Job drawing, mm, ordinate dimensions from the low corner. One solid piece. A direction names the side the tool comes from. Give positions to 0.01 mm unless a question says otherwise; leave off trailing zeros. Loops run counter-clockwise (first coordinate to the right, second up) from the corner with the lowest first, then second, coordinate; pieces in that order, holes last. Notation, with made-up numbers: (31, -27) -> (74, -27) arc R15 cw to (74, -9) -> close; hole circle Ø6 at (55.25, 1.25). An arc over 180 degrees is marked (long way). Use one line per item in the form item = value.
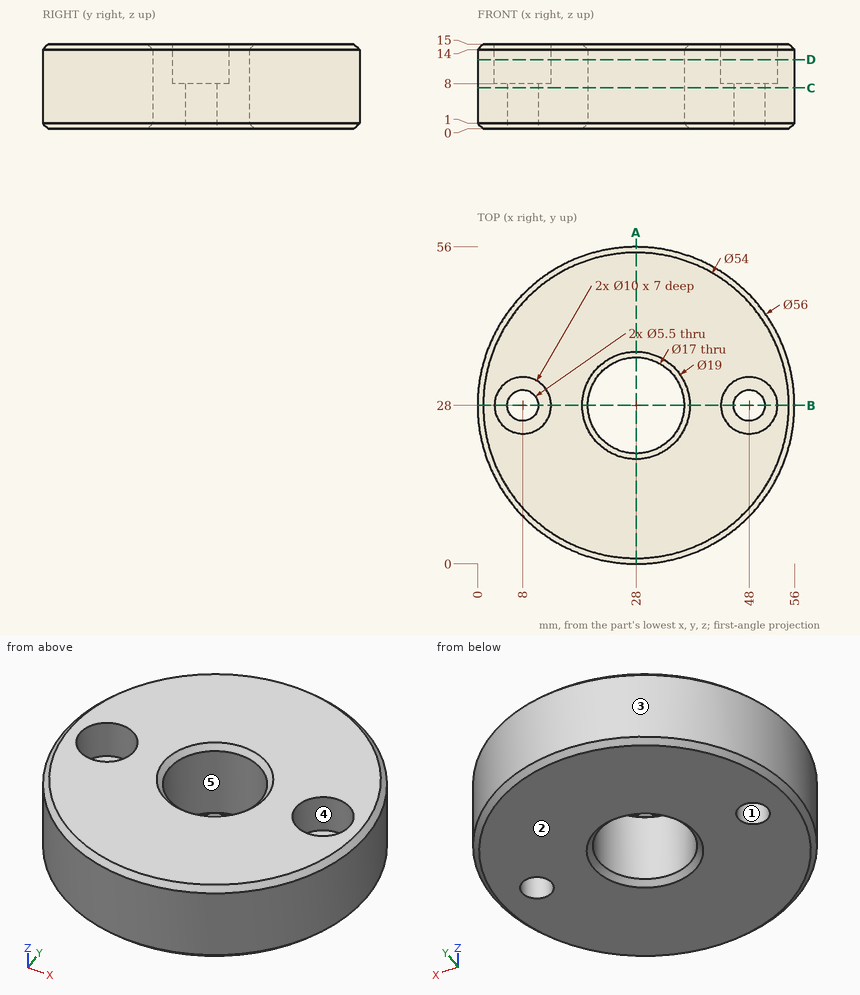
1. Cut at A-A, the plane x = 28. Write the cut outline in (y, z), then the cut area to 3 significant figures.
Result sheet:
outline = (0, 1) -> (1, 0) -> (18.5, 0) -> (19.5, 1) -> (19.5, 14) -> (18.5, 15) -> (1, 15) -> (0, 14) -> close; (36.5, 1) -> (37.5, 0) -> (55, 0) -> (56, 1) -> (56, 14) -> (55, 15) -> (37.5, 15) -> (36.5, 14) -> close
area = 581 mm^2
2. Drop flat-ended pins along their axis: P1, Ø4, axis at y = 41.5, z = 11, coming from the +X side; P2, Ø4, axis at x = 43.5, z = 8, coming from the +Y side; P3, Ø4, axis at y = 18.5, z = 13.5, coming from the -X side. Give the stop position or say it passes through.
Result sheet:
P1 = 53.53
P2 = 52.53
P3 = 1.02
3. Cut at B-B, the plane y = 28. State how many separate pieces and enclosed holes the cut face has, then the cut area to 3 significant figures.
Result sheet:
separate_pieces = 4
enclosed_holes = 0
area = 353 mm^2
4. Mould opens along Y. For the marked faces 1, 2 and 3 say: pulls with the +Y half, pulls with the -Y half, needs draft (parallel to the pull), parting line crosses it, or undercut.
Result sheet:
face_1 = undercut
face_2 = needs draft
face_3 = parting line crosses it
5. Cut at C-C, the plane z = 7.25. Write the cut outline in (x, y).
Result sheet:
outline = circle Ø56 at (28, 28); hole circle Ø5.5 at (8, 28); hole circle Ø17 at (28, 28); hole circle Ø5.5 at (48, 28)
6. Tool access for the marked faces 4 and 5: list every direction of +Z, -Z, +X, -X, +Y, -Y with a clear straight run to the whole face (end or side of a thin tool).
Result sheet:
face_4 = +Z
face_5 = +Z, -Z
7. Cut at D-D, the plane z = 12.25. Write the cut outline in (x, y).
Result sheet:
outline = circle Ø56 at (28, 28); hole circle Ø10 at (8, 28); hole circle Ø17 at (28, 28); hole circle Ø10 at (48, 28)
8. Drill centre lines: line 1 (Y direction, x = 28, z = 10); line 2 (X direction, y = 22.5, z = 14); line 3 (Y direction, x = 6.5, z = 3). Where is each one in solid material? Low to high.
Result sheet:
line_1 = 0 to 19.5, 36.5 to 56
line_2 = 0.55 to 21.52, 34.48 to 55.45
line_3 = 10.06 to 25.7, 30.3 to 45.94
